Build history of the part. All positions in model axes, mm. A direction names the side the tool comes from. Coordinates: 2 decimals unless noted, no trailing zeros. Order: outer loops, then holes, each group sorted by start corner. A loop starts at its lowest first (then second) coordinate and runs counter-clockwise, first axis right, second up. Notation, with made-up numbers: M -33.5,-22 L 11.5,-22 A22 ccw 11.5,15 Z; hole C -12,-30.5 d8. An arc over 180 degrees is marked long. Use a Markdown table: item, result. Add a question column.
from build123d import *

# Parameters (mm, degrees)
BASE_PLATE_SKETCH_W       = 90
BASE_PLATE_SKETCH_H       = 18
BASE_PLATE_90X18X50_DEPTH = 50
PIVOT_LUG_SKETCH_R        = 12
PIVOT_LUG_DEPTH           = 20
BOTTOM_GROOVE_SKETCH_W    = 20
BOTTOM_GROOVE_SKETCH_H    = 8
BOTTOM_GROOVE_DEPTH       = 120.163752878
LUG_START                 = -8
LUG_SLOT_DEPTH            = 8
TOP_POCKET_SKETCH_W       = 30
TOP_POCKET_SKETCH_H       = 15
TOP_POCKET_DEPTH          = 8
POCKET_HOLE_20_SKETCH_R   = 10
POCKET_HOLE_20_DEPTH      = 115.455231423


with BuildPart() as part:
    # Base Plate Sketch → Base Plate 90x18x50 (new body)
    with BuildSketch(Plane.XY):
        with Locations((45, 9)):
            Rectangle(BASE_PLATE_SKETCH_W, BASE_PLATE_SKETCH_H)
    extrude(amount=BASE_PLATE_90X18X50_DEPTH)

    # Pivot Lug Sketch → Pivot Lug (add)
    with BuildSketch(Plane.XY):
        with BuildLine():
            Line((20, 35), (20, 18))
            Line((20, 18), (70, 18))
            Line((70, 18), (70, 35))
            ThreePointArc((70, 35), (45, 60), (20, 35))
        make_face()
        with Locations((45, 35)):
            Circle(PIVOT_LUG_SKETCH_R, mode=Mode.SUBTRACT)
    extrude(amount=PIVOT_LUG_DEPTH)

    # Bottom Groove Sketch → Bottom Groove (cut, through all)
    with BuildSketch(Plane(origin=(90, 0, 0), x_dir=(0, 0, -1), z_dir=(1, 0, 0))):
        with Locations((-25, 4)):
            Rectangle(BOTTOM_GROOVE_SKETCH_W, BOTTOM_GROOVE_SKETCH_H)
    extrude(amount=-BOTTOM_GROOVE_DEPTH, mode=Mode.SUBTRACT)

    # Lug Slot Sketch → Lug Slot (cut)
    with BuildSketch(Plane.XY.offset(20).offset(LUG_START)):
        with BuildLine():
            Line((33, 35), (33, 56.931712199))
            ThreePointArc((33, 56.931712199), (45, 60), (57, 56.931712199))
            Line((57, 56.931712199), (57, 35))
            ThreePointArc((57, 35), (45, 47), (33, 35))
        make_face()
    extrude(amount=LUG_SLOT_DEPTH, mode=Mode.SUBTRACT)

    # Top Pocket Sketch → Top Pocket (cut)
    with BuildSketch(Plane(origin=(0, 18, 0), x_dir=(1, 0, 0), z_dir=(0, 1, 0))):
        with Locations((45, -42.5)):
            Rectangle(TOP_POCKET_SKETCH_W, TOP_POCKET_SKETCH_H)
    extrude(amount=-TOP_POCKET_DEPTH, mode=Mode.SUBTRACT)

    # Pocket Hole Ø20 Sketch → Pocket Hole Ø20 (cut, through all)
    with BuildSketch(Plane(origin=(0, 10, 0), x_dir=(1, 0, 0), z_dir=(0, 1, 0))):
        with Locations((45, -50)):
            Circle(POCKET_HOLE_20_SKETCH_R)
    extrude(amount=-POCKET_HOLE_20_DEPTH, mode=Mode.SUBTRACT)


solid = part.part
(1) Slice it at B-B on y = 4. Give the cut face in (x, z).
(2) Mould opens along Z. For faces 1 (the flat face through (46, 4, 15)), 2 (the flat face through (70, 26, 10)), 3 (the flat face through (72, 9, 50)) say: released by +Z, released by -Z, zero draft, split by the parting line, or undercut.
(3) Which spindle directions (+Z, -Z, +X, -X, +Y, -Y) get a long thin tool onto all of the face, cutting with end or side? Do faces 4 (the flat face through (20, 27, 10)), 5 (the flat face through (45, 50, 12)), 6 (the cylindrical face through (45.55, 59.994, 9.86)), 7 (the flat face through (46, 4, 35)). Say none if no direction does.
(4) Drill centre lines: line 1 along Y through (x, z) = (45, 10); line 2 along X through (y, z) = (35, 10); line 3 along Y through (x, z) = (6.5, 23.5). Where is each one in solid material? Low to high. Write a range as from..to.
(5) Drop flat-ended pins along their axis: P1, Ø19, axis at x = 40, y = 48.5, coming from the +Z side; P2, Ø2.5, axis at x = 38.5, y = 12.5, coming from the +Z side; P3, Ø1, axis at y = 36.5, z = 18, coming from the +X side. Give the stop position or say it passes through.
(6) Slice it at C-C on z = 4. Give the cut face in (x, y), and give its area (3 significant figures).
(7) Slice it at A-A on x = 45. Give the cut face in (y, z).
(8) Slice it at D-D on y = 48. Give the cut face in (x, z).
Solutions:
| question | item | result |
|---|---|---|
| 1 | outline | M 0,0 L 90,0 L 90,15 L 0,15 Z; M 0,35 L 90,35 L 90,50 L 55,50 A10 cw 35,50 L 0,50 Z |
| 2 | face 1 | undercut |
| 2 | face 2 | zero draft |
| 2 | face 3 | released by +Z |
| 3 | face 4 | +Z, -Z, -X, +Y |
| 3 | face 5 | +Z, +Y |
| 3 | face 6 | +Z, -Z, +Y |
| 3 | face 7 | +X, -X, -Y |
| 4 | line 1 | 0..23, 47..60 |
| 4 | line 2 | 20..33, 57..70 |
| 4 | line 3 | 8..18 |
| 5 | P1 | z = 20 |
| 5 | P2 | z = 35 |
| 5 | P3 | x = 69.98 |
| 6 | outline | M 0,0 L 90,0 L 90,18 L 70,18 L 70,35 A25 ccw 20,35 L 20,18 L 0,18 Z; hole C 45,35 d24 |
| 6 | area | 3,000 mm² |
| 7 | outline | M 0,0 L 23,0 L 23,20 L 18,20 L 18,35 L 10,35 L 10,40 L 0,40 L 0,35 L 8,35 L 8,15 L 0,15 Z; M 47,0 L 60,0 L 60,12 L 47,12 Z |
| 8 | outline | M 23.65,0 L 66.35,0 L 66.35,20 L 57,20 L 57,12 L 33,12 L 33,20 L 23.65,20 Z |
